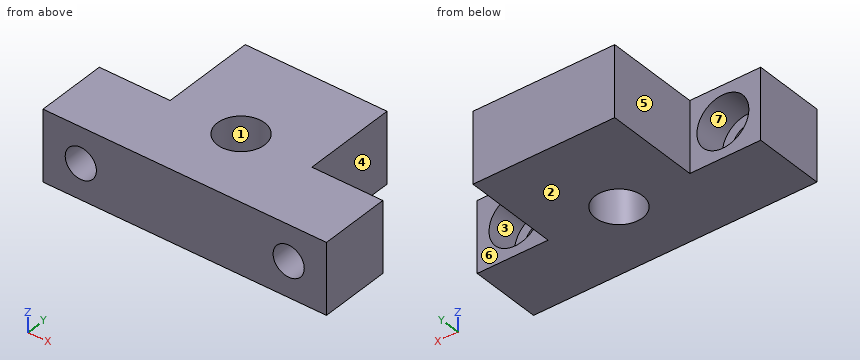
```python
from build123d import *

# Parameters (mm, degrees)
BOSS_EXTRUDE1_DEPTH                                  = 15
SKETCH2_R                                            = 5
CUT_EXTRUDE1_DEPTH                                   = 72.063352018
CBORE_FOR_M6_HEXAGON_SOCKET_HEAD_CAP_SCR_D           = 6.6
CBORE_FOR_M6_HEXAGON_SOCKET_HEAD_CAP_SCR_CBORE_D     = 11
CBORE_FOR_M6_HEXAGON_SOCKET_HEAD_CAP_SCR_CBORE_DEPTH = 6.8


with BuildPart() as part:
    # Sketch1 → Boss-Extrude1 (new body)
    with BuildSketch(Plane.XY):
        Polygon((0, 0), (0, 15), (15, 15), (15, 35), (45, 35), (45, 15), (60, 15), (60, 0), align=None)
    extrude(amount=BOSS_EXTRUDE1_DEPTH)

    # Sketch2 → Cut-Extrude1 (cut, through all)
    with BuildSketch(Plane.XY.offset(15)):
        with Locations((30, 15)):
            Circle(SKETCH2_R)
    extrude(amount=-CUT_EXTRUDE1_DEPTH, mode=Mode.SUBTRACT)

    # CBORE for M6 Hexagon socket head cap screws1 (through all)
    with Locations(Plane(origin=(8, 15, 7.5), x_dir=(0, 0, 1), z_dir=(0, 1, 0))):
        with Locations((0, 0), (0, 44)):
            CounterBoreHole(CBORE_FOR_M6_HEXAGON_SOCKET_HEAD_CAP_SCR_D / 2, CBORE_FOR_M6_HEXAGON_SOCKET_HEAD_CAP_SCR_CBORE_D / 2, CBORE_FOR_M6_HEXAGON_SOCKET_HEAD_CAP_SCR_CBORE_DEPTH)


solid = part.part
```
Input: part model. Units: mm. Frame: model coordinates. Face numbers are marked on the shaded views. A direction names the side the tool comes from. Give positions to 0.01 mm unless a question says otherwise; leave off trailing zeros. Order: outer loops, then holes, each group sorted by start corner. A loop starts at its lowest first (then second) coordinate and runs counter-clockwise, first axis right, second up. Notation, with made-up numbers: M 2,66.5 L 17,66.5 A18 ccw 17,87.5 Z; hole C 68.25,22 d1. An arc over 180 degrees is marked long. Return JSON: item names as keys, results as strings.
1) Section query D-D on y = 3. Output: boundary loops of the cut face in (x, z).
Taken from the geometry:
{"outline": "M 0,0 L 60,0 L 60,15 L 0,15 Z; hole C 8,7.5 d6.6; hole C 52,7.5 d6.6"}
2) Contact query for flat-ended pins moving along their axis: pin 1 (8 mm diameter, centred on y = 31, z = 12, fed in from +X); pin 2 (2 mm diameter, centred on x = 9, z = 9, fed in from +Y); pin 3 (7.5 mm diameter, centred on x = 6.5, z = 8, fed in from +Y); pin 4 (1.5 mm diameter, centred on y = 22, z = 8.5, fed in from -X). Output: stop coordinate, or through.
Taken from the geometry:
{"pin 1": "stops at x = 45", "pin 2": "passes through", "pin 3": "stops at y = 8.2", "pin 4": "stops at x = 15"}
3) Line query: L1, parallel to X at y = 3, z = 7.5; L2, parallel to X at y = 9.5, z = 7.5; L3, parallel to X at y = 12.5, z = 7.5. Output: solid intervals per line, ascending. Write a range as [from, to].
Taken from the geometry:
{"L1": "x = [0, 4.7], [11.3, 48.7], [55.3, 60]", "L2": "x = [0, 2.5], [13.5, 46.5], [57.5, 60]", "L3": "x = [0, 2.5], [13.5, 25.67], [34.33, 46.5], [57.5, 60]"}
4) Mould query, pull axis X, two halves, no side actions, for the marked faces 1, 2, 3 and 4. Classes: released by +X, released by -X, zero draft, split by the parting line, or undercut.
Taken from the geometry:
{"face 1": "undercut", "face 2": "zero draft", "face 3": "undercut", "face 4": "released by +X"}
5) Section query B-B on x = 30. Output: boundary loops of the cut face in (y, z).
Taken from the geometry:
{"outline": "M 0,0 L 10,0 L 10,15 L 0,15 Z; M 20,0 L 35,0 L 35,15 L 20,15 Z"}
6) Section query A-A on z = 7.5. Output: boundary loops of the cut face in (x, y).
Taken from the geometry:
{"outline": "M 0,0 L 4.7,0 L 4.7,8.2 L 2.5,8.2 L 2.5,15 L 0,15 Z; M 11.3,0 L 48.7,0 L 48.7,8.2 L 46.5,8.2 L 46.5,15 L 45,15 L 45,35 L 15,35 L 15,15 L 13.5,15 L 13.5,8.2 L 11.3,8.2 Z; M 55.3,0 L 60,0 L 60,15 L 57.5,15 L 57.5,8.2 L 55.3,8.2 Z; hole C 30,15 d10"}
7) Access query for the marked faces 5, 6 and 7. Directions: +Z, -Z, +X, -X, +Y, -Y. A direction counts if a zero-diameter tool reaches every point of the face in a straight line with its end or side. Return the directions, or none.
Taken from the geometry:
{"face 5": "+Z, -Z, -X, +Y", "face 6": "+Z, -Z, +X, +Y", "face 7": "+Y"}
8) Section query C-C on z = 1. Output: boundary loops of the cut face in (x, y).
Taken from the geometry:
{"outline": "M 0,0 L 60,0 L 60,15 L 45,15 L 45,35 L 15,35 L 15,15 L 0,15 Z; hole C 30,15 d10"}
